Input: part model. Units: mm. Frame: model coordinates. A direction names the side the tool comes from. Give positions to 0.01 mm unless a question says otherwise; leave off trailing zeros. Order: outer loops, then holes, each group sorted by start corner. A loop starts at its lowest first (then second) coordinate and runs counter-clockwise, first axis right, second up.
```python
from build123d import *

# Parameters (mm, degrees)
SKETCH1_W                    = 55
SKETCH1_H                    = 50
BOSS_EXTRUDE1_DEPTH          = 10
SKETCH4_W                    = 10
SKETCH4_H                    = 50
BOSS_EXTRUDE2_DEPTH          = 63
M8_CLEARANCE_HOLE1_D         = 9
M8_CLEARANCE_HOLE1_DEPTH     = 121
M8_CLEARANCE_HOLE1_TIP       = 2.703872786
CHAMFER1_SIZE                = 1
M14X1_5_TAPPED_HOLE1_D       = 12.5
CHAMFER2_SIZE                = 2
SIZE_MM_BLIND_DOWEL_HOLE_1_D = 6


with BuildPart() as part:
    # Sketch1 → Boss-Extrude1 (new body)
    with BuildSketch(Plane.XY):
        Rectangle(SKETCH1_W, SKETCH1_H)
    extrude(amount=BOSS_EXTRUDE1_DEPTH)

    # Sketch4 → Boss-Extrude2 (add)
    with BuildSketch(Plane(origin=(0, 0, 0), x_dir=(-1, 0, 0), z_dir=(0, 0, -1))):
        with Locations((-22.5, 0)):
            Rectangle(SKETCH4_W, SKETCH4_H)
    extrude(amount=BOSS_EXTRUDE2_DEPTH)

    # M8 Clearance Hole1
    with Locations(Plane(origin=(0, 0, 0), x_dir=(-1, 0, 0), z_dir=(0, 0, -1))):
        with Locations((17.5, -15), (17.5, 15), (-9.5, -15), (-9.5, 15)):
            Hole(M8_CLEARANCE_HOLE1_D / 2, depth=M8_CLEARANCE_HOLE1_DEPTH)
            with Locations((0, 0, -(M8_CLEARANCE_HOLE1_DEPTH + M8_CLEARANCE_HOLE1_TIP / 2))):  # 118° drill point
                Cone(0, M8_CLEARANCE_HOLE1_D / 2, M8_CLEARANCE_HOLE1_TIP, mode=Mode.SUBTRACT)

    # Chamfer1
    chamfer1_edges = [part.edges().sort_by_distance(p)[0] for p in [
        (-27.5, -25, 5),
        (-27.5, 25, 5),
    ]]
    chamfer(chamfer1_edges, length=CHAMFER1_SIZE)

    # M14x1.5 Tapped Hole1 (through all)
    with Locations(Plane(origin=(27.5, 0, 0), x_dir=(0, 0, -1), z_dir=(1, 0, 0))):
        with Locations((48, 0)):
            Hole(M14X1_5_TAPPED_HOLE1_D / 2)

    # Chamfer2
    chamfer2_edges = [part.edges().sort_by_distance(p)[0] for p in [
        (22.5, 25, -63),
        (22.5, -25, -63),
    ]]
    chamfer(chamfer2_edges, length=CHAMFER2_SIZE)

    # Size mm blind dowel hole 1 (through all)
    with Locations(Plane(origin=(0, 0, 0), x_dir=(-1, 0, 0), z_dir=(0, 0, -1))):
        with Locations((4, -15), (4, 15)):
            Hole(SIZE_MM_BLIND_DOWEL_HOLE_1_D / 2)


solid = part.part
```
1) Cut plane A-A (y = 15). Return the cut outline in (x, z).
2) Cut plane D-D (z = -56.5). Return the cut outline in (x, y), then the cut area to 3 significant figures.
3) Pull-direction query (Z, two-part tool) for faces 3 (the face through (22.43, 1.88, -42.04)), 4 (the face through (23, -24, -62)), 5 (the face through (11.919, 18.794, 5.07)); classes: pulls with the +Z half, pulls with the -Z half, needs draft (parallel to the pull), parting line crosses it, or undercut.
4) Cut plane C-C (x = -4). Return the cut outline in (y, z).
5) Line query: probe 1 along Y at (x, z) = (-4, 6.75); probe 2 along X at (y, z) = (-16, -38); probe 3 along Z at (x, y) = (-20, -23). Output: solid intervals per line, ascending.
6) Reachability of faces 1 (the face through (17.5, 0, -31)), 2 (the face through (-4.65, 12.07, 5.07)) from +Z, -Z, +X, -X, +Y, -Y: full face, straight path, thin tool, end or side. Return the list, or none.
7) First-contact query: P1, Ø22.5, axis at x = -1.5, y = 0, coming from the -Z side; P2, Ø25, axis at y = 1.5, z = -31.5, coming from the -X side; P3, Ø10.5, axis at x = 9.5, y = 15, coming from the +Z side. Flat tips, straight axial feed; report the tip coordinate or a pass-through.
8) Cut plane B-B (x = -17.5). Return the cut outline in (y, z), then the cut area to 3 significant figures.
Geometry says:
1. outline: (-27.5, 0) - (-22, 0) - (-22, 10) - (-27.5, 10) - close; (-13, 0) - (-7, 0) - (-7, 10) - (-13, 10) - close; (-1, 0) - (5, 0) - (5, 10) - (-1, 10) - close; (14, 0) - (17.5, 0) - (17.5, -63) - (27.5, -63) - (27.5, 10) - (14, 10) - close
2. outline: (17.5, -25) - (27.5, -25) - (27.5, 25) - (17.5, 25) - close
2. area: 500 mm2
3. face 3: undercut
3. face 4: pulls with the -Z half
3. face 5: needs draft
4. outline: (-25, 0) - (-18, 0) - (-18, 10) - (-25, 10) - close; (-12, 0) - (12, 0) - (12, 10) - (-12, 10) - close; (18, 0) - (25, 0) - (25, 10) - (18, 10) - close
5. probe 1: y = -25 to -18, -12 to 12, 18 to 25
5. probe 2: x = 17.5 to 27.5
5. probe 3: z = 0 to 10
6. face 1: -Z, -X, +Y, -Y
6. face 2: +Z, -Z
7. P1: stops at z = 0
7. P2: stops at x = 17.5
7. P3: stops at z = 10
8. outline: (-25, 0) - (-19.5, 0) - (-19.5, 10) - (-25, 10) - close; (-10.5, 0) - (10.5, 0) - (10.5, 10) - (-10.5, 10) - close; (19.5, 0) - (25, 0) - (25, 10) - (19.5, 10) - close
8. area: 320 mm2
